Can you work these out from the model? Positions are in its coordinate system, mm. A direction names the side the tool comes from. Coordinates: 2 decimals unless noted, no trailing zeros. Loops run counter-clockwise (first coordinate to the right, second up) from the corner with the lowest first, then second, coordinate; pieces in that order, holes last.
```python
from build123d import *

# Parameters (mm, degrees)
BOSS_EXTRUDE1_DEPTH = 15
BOSS_EXTRUDE2_START = 25.6
SKETCH5_R           = 15
BOSS_EXTRUDE2_DEPTH = 25.6
CHAMFER1_SIZE       = 1


with BuildPart() as part:
    # Sketch1 → Revolve1 (revolve)
    with BuildSketch(Plane.XY, mode=Mode.PRIVATE) as revolve1_sk:
        Polygon((35, 0), (60, 0), (60, 9.5), (59.5, 10), (60, 10.5), (60, 20), (42, 20), (21, 31), (15, 31), (15, 197), (0, 197), (0, 15), (14, 15), align=None)
    revolve(revolve1_sk.sketch.rotate(Axis((0, 197, 0), (0, -1, 0)), 180), axis=Axis((0, 197, 0), (0, -1, 0)))

    # Sketch2 → Boss-Extrude1 (add)
    with BuildSketch(Plane(origin=(0, 31, 0), x_dir=(1, 0, 0), z_dir=(0, 1, 0))):
        Polygon((15, 8.660254038), (0, 17.320508076), (-15, 8.660254038), (-15, -8.660254038), (0, -17.320508076), (15, -8.660254038), align=None)
    extrude(amount=BOSS_EXTRUDE1_DEPTH)

    # Sketch3 → Cut-Revolve1 (revolve, cut)
    with BuildSketch(Plane(origin=(0, 0, 0), x_dir=(0, 0, -1), z_dir=(1, 0, 0))):
        Polygon((15.820508076, 31), (17.320508076, 32.5), (17.320508076, 31), align=None)
        Polygon((17.320508076, 44.5), (15.820508076, 46), (17.320508076, 46), align=None)
    revolve(axis=Axis((0, 197, 0), (0, 1, 0)), mode=Mode.SUBTRACT)

    # Sketch5 → Boss-Extrude2 (add)
    with BuildSketch(Plane(origin=(0, 47, 0), x_dir=(-1, 0, 0), z_dir=(0, 1, 0)).offset(BOSS_EXTRUDE2_START)):
        Polygon((0, 26.558112383), (-23, 13.279056191), (-23, -13.279056191), (0, -26.558112383), (23, -13.279056191), (23, 13.279056191), align=None)
        Circle(SKETCH5_R, mode=Mode.SUBTRACT)
    extrude(amount=-BOSS_EXTRUDE2_DEPTH)

    # Sketch7 → Cut-Revolve3 (revolve, cut)
    with BuildSketch(Plane(origin=(0, 0, 0), x_dir=(0, 0, -1), z_dir=(1, 0, 0))):
        Polygon((23.858112383, 72.6), (26.558112383, 69.9), (26.558112383, 72.6), align=None)
        Polygon((23.858112383, 47), (26.558112383, 49.7), (26.558112383, 47), align=None)
    revolve(axis=Axis((0, 197, 0), (0, 1, 0)), mode=Mode.SUBTRACT)

    # Chamfer1
    chamfer1_edges = [part.edges().sort_by_distance(p)[0] for p in [
        (15, 197, 0),
    ]]
    chamfer(chamfer1_edges, length=CHAMFER1_SIZE)


solid = part.part
```
(1) If we mould it in two halves opening along X, with no side actions, what happens to faces 4 (the flat face through (15, 38, 0)), 5 (the flat face through (-7.4, 38.4, -13.05)), 6 (the flat face through (0, 15, 0))? For each: released by +X, released by -X, zero draft, split by the parting line, or undercut.
Check values:
face 4: released by +X
face 5: released by -X
face 6: undercut
(2) I want a section at A-A on y = 182.5. Write out the boundary of the cut face in (x, z).
Check values:
outline: circle Ø30 at (0, 0)
(3) Which directions (+Z, -Z, +X, -X, +Y, -Y) give clear straight access to the entire face, cutting with the end or side of a thin tool? Please do faces 1 (the flat face through (-11.34, 59.98, -20.01)), 2 (the flat face through (11, 72.6, 11)), 3 (the flat face through (13.2, 46, -7.5)).
Check values:
face 1: -Z, -X, +Y
face 2: +Y
face 3: -Z, +X
(4) If I drill on probe 1 along Y at (x, z) = (-22.5, -43.5); probe 2 along X at (y, z) = (69.5, -2.5); probe 3 along Y at (x, z) = (22, -12.5), over which ranges is the centre line in solid material (lowest first)?
Check values:
probe 1: y = 0 to 20
probe 2: x = -23 to 23
probe 3: y = 6.93 to 28.75, 48.45 to 71.15
(5) I want a section at B-B on y = 27.5. Write out the boundary of the cut face in (x, z).
Check values:
outline: circle Ø55.36 at (0, 0)
(6) I'm going to push flat-ended pins straight in: pin 1 (12 mm diameter, centred on y = 36, z = -4, fed in from -X); pin 2 (1 mm diameter, centred on x = 16, y = 66, fed in from -Z); pin 3 (4 mm diameter, centred on x = 15, z = -14.5, fed in from -Y). Where does each tip first touch, or does it pass through?
Check values:
pin 1: stops at x = -22.6
pin 2: stops at z = -17.61
pin 3: stops at y = 8.67
